Here's how the part is built. I have some questions about the finished solid (model axes, mm). A direction names the side the tool comes from. Round coordinates to 2 decimals unless told otherwise and drop trailing zeros. Loops run counter-clockwise (first coordinate to the right, second up) from the corner with the lowest first, then second, coordinate; pieces in that order, holes last. Notation, with made-up numbers: M -27,85 L 12,85 A10 ccw 12,92 Z; hole C 82,-14.75 d7. An arc over 180 degrees is marked long. Use a Markdown table: item, result.
```python
from build123d import *

# Parameters (mm, degrees)
G3_4_TAPPED_HOLE1_D     = 24.5
G3_4_TAPPED_HOLE1_DEPTH = 58.32
G3_4_TAPPED_HOLE1_TIP   = 7.360542583
CHAMFER1_SIZE           = 2


with BuildPart() as part:
    # Sketch1 → Revolve1 (revolve)
    with BuildSketch(Plane.XY, mode=Mode.PRIVATE) as revolve1_sk:
        Polygon((0, 0), (20, 0), (20, -12), (17.5, -12), (17.5, -20), (0, -20), align=None)
    revolve(revolve1_sk.sketch.rotate(Axis((0, -20, 0), (0, 1, 0)), 90), axis=Axis((0, -20, 0), (0, 1, 0)))

    # G3/4 Tapped Hole1
    with Locations(Plane(origin=(0, 0, 0), x_dir=(1, 0, 0), z_dir=(0, 1, 0))):
        with Locations((0, 0)):
            Hole(G3_4_TAPPED_HOLE1_D / 2, depth=G3_4_TAPPED_HOLE1_DEPTH)
            with Locations((0, 0, -(G3_4_TAPPED_HOLE1_DEPTH + G3_4_TAPPED_HOLE1_TIP / 2))):  # 118° drill point
                Cone(0, G3_4_TAPPED_HOLE1_D / 2, G3_4_TAPPED_HOLE1_TIP, mode=Mode.SUBTRACT)

    # Chamfer1
    chamfer1_edges = [part.edges().sort_by_distance(p)[0] for p in [
        (0, 0, 20),
    ]]
    chamfer(chamfer1_edges, length=CHAMFER1_SIZE)


solid = part.part
```
Q1. For faces 4 (the cylindrical face through (17.084, -16.056, 3.794)), 5 (the cylindrical face through (-0.88, -7.07, 19.98)), which set-ups out of +Z, -Z, +X, -X, +Y, -Y let a thin tool reach every point of the face, with its end or its side?
Return value:
| item | result |
|---|---|
| face 4 | -Y |
| face 5 | +Y, -Y |
Q2. I need wall thicknesses on line 1 (Y direction, x = -17, z = -4.5); line 2 (Z direction, x = -5.5, y = -16.75); line 3 (Z direction, x = -1.5, y = -16). Which ranges of each line are inside material? Lowest first, please. Write a range as from..to.
Return value:
| item | result |
|---|---|
| line 1 | y = -12..0 |
| line 2 | z = -16.61..-10.95, 10.95..16.61 |
| line 3 | z = -17.44..-12.16, 12.16..17.44 |
Q3. Will these pins go through, and if not, where does the flat tip stop? P1, Ø1.5, axis at x = 15.5, z = 15, coming from the -Y side; P2, Ø2, axis at y = -3.5, z = 6, coming from the -X side; P3, Ø3, axis at x = 5, y = -7.5, coming from the -Z side; P4, Ø12, axis at y = -5.5, z = 16, coming from the -X side.
Return value:
| item | result |
|---|---|
| P1 | passes through |
| P2 | stops at x = -19.36 |
| P3 | stops at z = -19.69 |
| P4 | stops at x = -17.32 |
Q4. Imagine slicing it at B-B, the plane x = 0. Please give me the cut outline in (y, z), then the cut area to 3 significant figures.
Return value:
| item | result |
|---|---|
| outline | M -20,-17.5 L -12,-17.5 L -12,-20 L -2,-20 L 0,-18 L 0,-12.25 L -20,-12.25 Z; M -20,12.25 L 0,12.25 L 0,18 L -2,20 L -12,20 L -12,17.5 L -20,17.5 Z |
| area | 266 mm^2 |
Q5. Imagine slicing it at A-A, the plane z = 0. Please give me the cut outline in (x, y), then the cut area to 3 significant figures.
Return value:
| item | result |
|---|---|
| outline | M -20,-12 L -17.5,-12 L -17.5,-20 L -12.25,-20 L -12.25,0 L -18,0 L -20,-2 Z; M 12.25,-20 L 17.5,-20 L 17.5,-12 L 20,-12 L 20,-2 L 18,0 L 12.25,0 Z |
| area | 266 mm^2 |
Q6. Imagine slicing it at C-C, the plane y = -7. Please give me the cut outline in (x, z), then the cut area to 3 significant figures.
Return value:
| item | result |
|---|---|
| outline | C 0,0 d40; hole C 0,0 d24.5 |
| area | 785 mm^2 |
Q7. We'd pull the mould along X, two halves only. Please class faces 1 (the cylindrical face through (-6.586, -10.14, -10.329)), 2 (the flat face through (12, 0, 4)), 3 (the conical face through (-5.444, -0.125, -17.288)): pulls with the +X half, pulls with the -X half, needs draft (parallel to the pull), parting line crosses it, or undercut.
Return value:
| item | result |
|---|---|
| face 1 | undercut |
| face 2 | needs draft |
| face 3 | parting line crosses it |
